Part model, mm, in its own coordinate system. A direction names the side the tool comes from. Coordinates: 2 decimals unless noted, no trailing zeros. Write each loop counter-clockwise with the first axis right and the second up, starting at its lowest first coordinate (ties: lowest second). Pieces come first, ordered by that corner, then holes. Notation, with made-up numbers: M 23,-18.5 L 35,-18.5 A25 cw 35,9.5 Z; hole C -14,87 d1. An arc over 180 degrees is marked long. Use a Markdown table: item, result. Add a question column.
Q1. Slice it at A-A on x = 0. Write the cut outline in (y, z).
Q2. Tool access for faces 4 (the flat face through (-25, 0, 12)), 5 (the flat face through (4, -4, 21)): list every direction of +Z, -Z, +X, -X, +Y, -Y with a clear straight run to the whole face (end or side of a thin tool).
Q3. Pin check, flat tip, straight feed: pin 1 Ø16 at (x, y) = (3, 5) entering from +Z. Stop position of the tip, or through.
Q4. Wall check: L1, parallel to Y at x = 0, z = 6.25; L2, parallel to Z at x = -7, y = 0.5; L3, parallel to Y at x = 0, z = 26. Give the ranges that are in metal, low to high. Write a range as from..to.
Q5. Mould opens along X. For faces 1 (the flat face through (-17, 11, 24)), 2 (the cylindrical face through (-4.336, -19.524, 26.028)), 3 (the cylindrical face through (-5, 1.6, 10.4)) say: released by +X, released by -X, zero draft, split by the parting line, or undercut.
from build123d import *

# Parameters (mm, degrees)
SKETCH_1_W          = 50
SKETCH_1_H          = 50
EXTRUDE_1_DEPTH     = 29
SKETCH_3_R          = 10
CUT_EXTRUDE_1_DEPTH = 8
SKETCH_4_R          = 5.25
CUT_EXTRUDE_2_DEPTH = 21
CHAMFER_1_SIZE      = 1
SKETCH_5_OUTSIDE_W  = 67.286
SKETCH_5_OUTSIDE_H  = 67.286
SKETCH_5_OUTSIDE_R  = 20
CUT_EXTRUDE_3_DEPTH = 5
CHAMFER_2_SIZE      = 1


with BuildPart() as part:
    # 草图1 → 凸台-拉伸1 (new body)
    with BuildSketch(Plane.XY):
        Rectangle(SKETCH_1_W, SKETCH_1_H)
    extrude(amount=EXTRUDE_1_DEPTH)

    # 草图3 → 切除-拉伸1 (cut)
    with BuildSketch(Plane.XY.offset(29)):
        Circle(SKETCH_3_R)
    extrude(amount=-CUT_EXTRUDE_1_DEPTH, mode=Mode.SUBTRACT)

    # 草图4 → 切除-拉伸2 (cut)
    with BuildSketch(Plane(origin=(0, 0, 0), x_dir=(-1, 0, 0), z_dir=(0, 0, -1))):
        Circle(SKETCH_4_R)
    extrude(amount=-CUT_EXTRUDE_2_DEPTH, mode=Mode.SUBTRACT)

    # 倒角1
    chamfer_1_edges = [part.edges().sort_by_distance(p)[0] for p in [
        (-10, 0, 29),
    ]]
    chamfer(chamfer_1_edges, length=CHAMFER_1_SIZE)

    # 草图5 outside → 切除-拉伸3 (cut)
    with BuildSketch(Plane.XY.offset(29)):
        Rectangle(SKETCH_5_OUTSIDE_W, SKETCH_5_OUTSIDE_H)
        Circle(SKETCH_5_OUTSIDE_R, mode=Mode.SUBTRACT)
    extrude(amount=-CUT_EXTRUDE_3_DEPTH, mode=Mode.SUBTRACT)

    # 倒角2
    chamfer_2_edges = [part.edges().sort_by_distance(p)[0] for p in [
        (-20, 0, 29),
    ]]
    chamfer(chamfer_2_edges, length=CHAMFER_2_SIZE)


solid = part.part
Recorded:
| question | item | result |
|---|---|---|
| 1 | outline | M -25,0 L -5.25,0 L -5.25,21 L -10,21 L -10,28 L -11,29 L -19,29 L -20,28 L -20,24 L -25,24 Z; M 5.25,0 L 25,0 L 25,24 L 20,24 L 20,28 L 19,29 L 11,29 L 10,28 L 10,21 L 5.25,21 Z |
| 2 | face 4 | +Z, -Z, -X, +Y, -Y |
| 2 | face 5 | +Z |
| 3 | pin 1 | z = 29 |
| 4 | L1 | -25..-5.25, 5.25..25 |
| 4 | L2 | 0..21 |
| 4 | L3 | -20..-10, 10..20 |
| 5 | face 1 | zero draft |
| 5 | face 2 | split by the parting line |
| 5 | face 3 | undercut |
